from build123d import *

# Parameters (mm, degrees)
SIZE_MM_DOWEL_HOLE1_D           = 2
SIZE_MM_DOWEL_HOLE1_DEPTH       = 2.5
SIZE_MM_DOWEL_HOLE1_CSINK_D     = 2.5
SIZE_MM_DOWEL_HOLE1_CSINK_ANGLE = 90
SIZE_MM_DOWEL_HOLE1_TIP         = 0.600860619
CUT_EXTRUDE1_DEPTH              = 2.5


with BuildPart() as part:
    # Sketch2 → Revolve1 (revolve)
    with BuildSketch(Plane(origin=(0, 0, 0), x_dir=(1, 0, 0), z_dir=(0, 1, 0))):
        Polygon((0, 0), (2.7, 0), (2.9, 0.2), (2.9, 0.8), (2.7, 1), (2, 1), (2, 12.2), (1.2, 12.2), (1.2, 12.4), (1.5, 12.7), (1.5, 18), (1.3, 18.2), (0, 18.2), align=None)
    revolve(axis=Axis((0, 0, 4.425925926), (0, 0, -1)))

    # Size mm Dowel Hole1
    with Locations(Plane.XY):
        with Locations((0, 0)):
            CounterSinkHole(SIZE_MM_DOWEL_HOLE1_D / 2, SIZE_MM_DOWEL_HOLE1_CSINK_D / 2, depth=SIZE_MM_DOWEL_HOLE1_DEPTH, counter_sink_angle=SIZE_MM_DOWEL_HOLE1_CSINK_ANGLE)
            with Locations((0, 0, -(SIZE_MM_DOWEL_HOLE1_DEPTH + SIZE_MM_DOWEL_HOLE1_TIP / 2))):  # 118° drill point
                Cone(0, SIZE_MM_DOWEL_HOLE1_D / 2, SIZE_MM_DOWEL_HOLE1_TIP, mode=Mode.SUBTRACT)

    # Sketch5 → Cut-Extrude1 (cut)
    with BuildSketch(Plane.XY):
        Polygon((0.577350269, -1), (1.154700538, 0), (0.577350269, 1), (-0.577350269, 1), (-1.154700538, 0), (-0.577350269, -1), align=None)
    extrude(amount=-CUT_EXTRUDE1_DEPTH, mode=Mode.SUBTRACT)


solid = part.part
Read the model definition and answer for the solid it produces. Units are mm, in the model's axes. A direction names the side the tool comes from. Round coordinates to 2 decimals unless told otherwise and drop trailing zeros. Write each loop counter-clockwise with the first axis right and the second up, starting at its lowest first coordinate (ties: lowest second). Pieces come first, ordered by that corner, then holes.
Q1. Flat-ended cylindrical pins translate along their axes: P1, Ø1.5, axis at x = 1, z = -9.5, coming from the +Y side; P2, Ø0.9, axis at x = 0, z = -1.5, coming from the -Y side; P3, Ø2, axis at x = 0, z = -14.5, coming from the +Y side. Find the tip coordinate at first contact, or state that the pin passes through.
Values:
P1: stops at y = 1.98
P2: stops at y = -2
P3: stops at y = 1.5
Q2. Find section A-A on z = -8.5. Determine the outline of the cut face in (x, y), and give its area (3 significant figures).
Values:
outline: circle Ø4 at (0, 0)
area: 12.6 mm2
Q3. A tool of negligible diameter and unlimited length cuts with its end or side. For faces 1 (the face through (-1, 1, 0)), 2 (the face through (-0.86, 0.51, -1.28)), 3 (the face through (0, 2, -7)), from which of +Z, -Z, +X, -X, +Y, -Y can it reach the whole face along a straight path? Write none if from no direction.
Values:
face 1: +Z, +X, -X, +Y, -Y
face 2: +Z
face 3: -Z
Q4. The mould has two halves that part along Z. Classify faces 4 (the face through (1, 1, -12.2)), 5 (the face through (-2, 1, -1)), 6 (the face through (0.86, -0.51, -1.28)): released by +Z, released by -Z, zero draft, split by the parting line, or undercut.
Values:
face 4: undercut
face 5: released by -Z
face 6: zero draft
Q5. Find section B-B on z = -14.75. Determine the outline of the cut face in (x, y).
Values:
outline: circle Ø3 at (0, 0)
Q6. Straight lines are drawn through the part: line 1 (Z direction, x = -1.35, y = 1.7); line 2 (Z direction, x = -0.95, y = 1.3); line 3 (Y direction, x = -0.25, z = -7.5). For each, find the intervals that lie inside material, in ascending order.
Values:
line 1: z = -1 to 0
line 2: z = -12.2 to 0
line 3: y = -1.98 to 1.98
